from build123d import *

# Parameters (mm, degrees)
CUT_EXTRUDE_1_DEPTH = 5
SKETCH_3_R          = 20
SKETCH_3_R_2        = 18.75
CUT_EXTRUDE_2_DEPTH = 1.7


with BuildPart() as part:
    # 草图1 → 旋转1 (revolve)
    with BuildSketch(Plane.XY):
        Polygon((0, 0), (0, 22.5), (58, 22.5), (58, 25), (978, 25), (978, 22.5), (1076, 22.5), (1076, 20), (1162, 20), (1162, 0), align=None)
    revolve(axis=Axis((1162, 0, 0), (-1, 0, 0)))

    # 草图2 → 切除-拉伸1 (cut)
    with BuildSketch(Plane(origin=(0, 20, 0), x_dir=(1, 0, 0), z_dir=(0, 1, 0))):
        with BuildLine():
            Line((1086, 6), (1172, 6))
            Line((1172, 6), (1172, -6))
            Line((1172, -6), (1086, -6))
            ThreePointArc((1086, -6), (1080, 0), (1086, 6))
        make_face()
    extrude(amount=-CUT_EXTRUDE_1_DEPTH, mode=Mode.SUBTRACT)

    # 草图3 → 切除-拉伸2 (cut)
    with BuildSketch(Plane(origin=(1151.5, 0, 0), x_dir=(0, 0, -1), z_dir=(1, 0, 0))):
        with Locations(Location((0, 0, 0), (0, 0, 90))):
            Circle(SKETCH_3_R)
        Circle(SKETCH_3_R_2, mode=Mode.SUBTRACT)
    extrude(amount=-CUT_EXTRUDE_2_DEPTH, mode=Mode.SUBTRACT)


solid = part.part
Geometry check sheet. Reference: the model listing, model coordinates, mm. A direction names the side the tool comes from. Coordinates: 2 decimals unless noted, no trailing zeros. Order: outer loops, then holes, each group sorted by start corner. A loop starts at its lowest first (then second) coordinate and runs counter-clockwise, first axis right, second up. Notation, with made-up numbers: M 9,33.5 L 63,33.5 A23 ccw 63,43.5 Z; hole C 12.25,21 d11. An arc over 180 degrees is marked long. Use CSV: the item, a comma, the result in double quotes.
Item 1: Cross-section at A-A on y = 0. Record the cut outline in (x, z).
Returned:
outline,"M 0,-22.5 L 58,-22.5 L 58,-25 L 978,-25 L 978,-22.5 L 1076,-22.5 L 1076,-20 L 1149.8,-20 L 1149.8,-18.75 L 1151.5,-18.75 L 1151.5,-20 L 1162,-20 L 1162,20 L 1151.5,20 L 1151.5,18.75 L 1149.8,18.75 L 1149.8,20 L 1076,20 L 1076,22.5 L 978,22.5 L 978,25 L 58,25 L 58,22.5 L 0,22.5 Z"
Item 2: Gauge pin test, flat ends, axial feed: pin 1 Ø1.2 at (x, y) = (1134, 16.5) entering from -Z; pin 2 Ø6 at (x, y) = (810.5, 9.5) entering from -Z; pin 3 Ø8 at (x, z) = (762, -8.5) entering from -Y. Record the tip position at first contact, or that the pin passes through.
Returned:
pin 1,"stops at z = -12.13"
pin 2,"stops at z = -24.14"
pin 3,"stops at y = -24.59"
Item 3: Mould release check, pull along X, two halves, no side actions. Record for faces 6 (the cylindrical face through (1027.686, 10.382, 19.961)), 7 (the flat face through (1149.8, -18, -6)), 8 (the flat face through (1076, -20.1, 1.6)), 9 (the flat face through (1151.5, -18, -6)): pulls with the +X half, pulls with the -X half, needs draft (parallel to the pull), parting line crosses it, or undercut.
Returned:
face 6,"needs draft"
face 7,"undercut"
face 8,"pulls with the +X half"
face 9,"undercut"
Item 4: Tool access check on faces 1 (the flat face through (0, 0, 0)), 2 (the flat face through (58, 22.34, -3.82)), 3 (the flat face through (1162, -1, 0)), 4 (the cylindrical face through (1150.662, -18.735, 0.739)), 5 (the cylindrical face through (1113.417, -4.336, 19.524)). Record the directions out of +Z, -Z, +X, -X, +Y, -Y that give a thin tool (end or side, any length) a straight path to the whole face; none if there is none.
Returned:
face 1,"+Z, -Z, -X, +Y, -Y"
face 2,"-X"
face 3,"+Z, -Z, +X, +Y, -Y"
face 4,"none"
face 5,"+X"
Item 5: Thickness scan on line 1 along X through (y, z) = (-14, -13.5); line 2 along Z through (x, y) = (272, -1); line 3 along Y through (x, z) = (145.5, -16.5). Record the ranges inside material, lowest first.
Returned:
line 1,"x = 0 to 1149.8, 1151.5 to 1162"
line 2,"z = -24.98 to 24.98"
line 3,"y = -18.78 to 18.78"
Item 6: Cross-section at B-B on x = 687. Record the cut outline in (y, z), then the cut area to 3 significant figures.
Returned:
outline,"C 0,0 d50"
area,"1,960 mm2"
